Can you work these out from the drawing? Everything is in mm from the part's minimum corner. Coordinates: 2 decimals unless noted, no trailing zeros. Write each loop counter-clockwise with the first axis right and the second up, starting at its lowest first coordinate (ties: lowest second). Pieces come first, ordered by that corner, then holes.
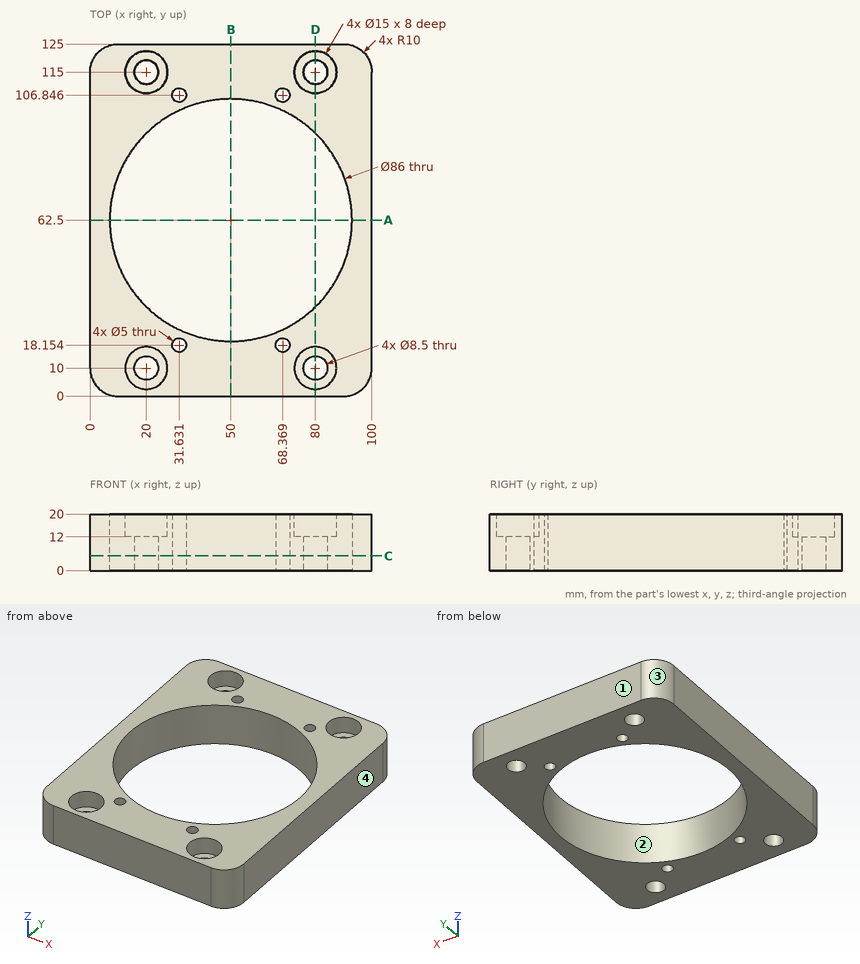
1. I want a section at B-B (x = 50). List the corners of the cut face in (y, z) for me.
2. If I drill on line 1 (X direction, y = 114.5, z = 12.5); line 2 (Y direction, x = 50, z = 11); line 3 (Y direction, x = 18.5, z = 4.75), over which ranges is the centre line in solid material (lowest first)?
3. I want a section at D-D (x = 80). List the corners of the cut face in (y, z) for me.
4. I want a section at C-C (z = 5.25). State how many separate pieces and enclosed holes the cut face has, then the cut area to 3 significant figures.
5. I want a section at A-A (y = 62.5). List the corners of the cut face in (x, z) for me, then the cut area to 3 significant figures.
6. Thinking about a two-plate mould opening in X: for the marked faces 1, 2, 3 and 4, which applies, pulls with the +X half, pulls with the -X half, needs draft (parallel to the pull), parting line crosses it, or undercut?
7. For pin 1 Ø10 at (x, y) = (80, 10) entering from +Z; pin 2 Ø7 at (x, y) = (20, 10) entering from -Z, each with a flat end and sliding along its axis, tell me the tip position at first contact or that it passes through.
Response values:
1. outline: (0, 0) - (19.5, 0) - (19.5, 20) - (0, 20) - close; (105.5, 0) - (125, 0) - (125, 20) - (105.5, 20) - close
2. line 1: x = 0 to 12.52, 27.48 to 72.52, 87.48 to 100
2. line 2: y = 0 to 19.5, 105.5 to 125
2. line 3: y = 0 to 6.02, 13.98 to 33.23, 91.77 to 111.02, 118.98 to 125
3. outline: (0, 0) - (5.75, 0) - (5.75, 12) - (2.5, 12) - (2.5, 20) - (0, 20) - close; (14.25, 0) - (31.69, 0) - (31.69, 20) - (17.5, 20) - (17.5, 12) - (14.25, 12) - close; (93.31, 0) - (110.75, 0) - (110.75, 12) - (107.5, 12) - (107.5, 20) - (93.31, 20) - close; (119.25, 0) - (125, 0) - (125, 20) - (122.5, 20) - (122.5, 12) - (119.25, 12) - close
4. separate pieces: 1
4. enclosed holes: 9
4. area: 6,300 mm2
5. outline: (0, 0) - (7, 0) - (7, 20) - (0, 20) - close; (93, 0) - (100, 0) - (100, 20) - (93, 20) - close
5. area: 280 mm2
6. face 1: needs draft
6. face 2: undercut
6. face 3: pulls with the -X half
6. face 4: pulls with the +X half
7. pin 1: stops at z = 12
7. pin 2: passes through
